```python
from build123d import *

# Parameters (mm, degrees)
SKETCH1_W                       = 100
SKETCH1_H                       = 270
BOSS_EXTRUDE1_DEPTH             = 20
M8_TAPPED_HOLE1_D               = 6.8
M8_TAPPED_HOLE1_DEPTH           = 19.75
M8_TAPPED_HOLE1_TIP             = 2.042926105
M8_TAPPED_HOLE1_ON_FACE_2_D     = 6.8
M8_TAPPED_HOLE1_ON_FACE_2_DEPTH = 19.75
M8_TAPPED_HOLE1_ON_FACE_2_TIP   = 2.042926105
M4_TAPPED_HOLE2_D               = 3.3
M4_TAPPED_HOLE2_DEPTH           = 10.1
M4_TAPPED_HOLE2_TIP             = 0.991420021
M4_TAPPED_HOLE1_D               = 3.3
M4_TAPPED_HOLE1_DEPTH           = 10.1
M4_TAPPED_HOLE1_TIP             = 0.991420021


with BuildPart() as part:
    # Sketch1 → Boss-Extrude1 (new body)
    with BuildSketch(Plane.XY):
        with Locations((50, -135)):
            Rectangle(SKETCH1_W, SKETCH1_H)
    extrude(amount=BOSS_EXTRUDE1_DEPTH)

    # M8 Tapped Hole1
    with Locations(Plane(origin=(15, 0, 10), x_dir=(0, 0, 1), z_dir=(0, 1, 0))):
        with Locations((0, 0), (0, 70)):
            Hole(M8_TAPPED_HOLE1_D / 2, depth=M8_TAPPED_HOLE1_DEPTH)
            with Locations((0, 0, -(M8_TAPPED_HOLE1_DEPTH + M8_TAPPED_HOLE1_TIP / 2))):  # 118° drill point
                Cone(0, M8_TAPPED_HOLE1_D / 2, M8_TAPPED_HOLE1_TIP, mode=Mode.SUBTRACT)

    # M8 Tapped Hole1 on face 2
    with Locations(Plane(origin=(15, -270, 10), x_dir=(0, 0, -1), z_dir=(0, -1, 0))):
        with Locations((0, 0), (0, 70)):
            Hole(M8_TAPPED_HOLE1_ON_FACE_2_D / 2, depth=M8_TAPPED_HOLE1_ON_FACE_2_DEPTH)
            with Locations((0, 0, -(M8_TAPPED_HOLE1_ON_FACE_2_DEPTH + M8_TAPPED_HOLE1_ON_FACE_2_TIP / 2))):  # 118° drill point
                Cone(0, M8_TAPPED_HOLE1_ON_FACE_2_D / 2, M8_TAPPED_HOLE1_ON_FACE_2_TIP, mode=Mode.SUBTRACT)

    # M4 Tapped Hole2
    with Locations(Plane.XY.offset(20)):
        with Locations((50, -127.5), (50, -142.5)):
            Hole(M4_TAPPED_HOLE2_D / 2, depth=M4_TAPPED_HOLE2_DEPTH)
            with Locations((0, 0, -(M4_TAPPED_HOLE2_DEPTH + M4_TAPPED_HOLE2_TIP / 2))):  # 118° drill point
                Cone(0, M4_TAPPED_HOLE2_D / 2, M4_TAPPED_HOLE2_TIP, mode=Mode.SUBTRACT)

    # M4 Tapped Hole1
    with Locations(Plane(origin=(0, 0, 0), x_dir=(-1, 0, 0), z_dir=(0, 0, -1))):
        with Locations((-60, -55), (-60, -115), (-60, -175)):
            Hole(M4_TAPPED_HOLE1_D / 2, depth=M4_TAPPED_HOLE1_DEPTH)
            with Locations((0, 0, -(M4_TAPPED_HOLE1_DEPTH + M4_TAPPED_HOLE1_TIP / 2))):  # 118° drill point
                Cone(0, M4_TAPPED_HOLE1_D / 2, M4_TAPPED_HOLE1_TIP, mode=Mode.SUBTRACT)


solid = part.part
```
Work out the finished part from the listing and answer in its coordinate system (mm). A direction names the side the tool comes from. Round coordinates to 2 decimals unless told otherwise and drop trailing zeros. Return JSON: item names as keys, results as strings. Group by question number.
Q1. Find the intervals of material crossed by L1, parallel to X at y = -14.75, z = 10; L2, parallel to Y at x = 50, z = 17; L3, parallel to X at y = -127.5, z = 17.5, in increasing order.
Q2. For faces 1 (the flat face through (49, -133, 0)), 2 (the cylindrical face through (81.68, -10.01, 10.74)), 3 (the cylindrical face through (81.68, -259.99, 9.26)), determine the directions among +Z, -Z, +X, -X, +Y, -Y from which every point of the face is accessible in a straight line to the end or side of a thin tool.
Q3. Each of these flat-tipped pins is pushed along its axis until it touches: pin 1 Ø4 at (x, z) = (85, 10) entering from -Y; pin 2 Ø6 at (x, z) = (15, 10) entering from -Y; pin 3 Ø2.5 at (x, y) = (60, -175) entering from -Z. Where does it stop, or does it pass through?
Q4. The mould has two halves that part along X. Classify faces 4 (the flat face through (49, -133, 20)), 5 (the cylindrical face through (12, -10, 8.4)), 6 (the flat face through (100, -137, 10)): released by +X, released by -X, zero draft, split by the parting line, or undercut.
Solved:
{
 "1": {"L1": "0 to 11.6, 18.4 to 81.6, 88.4 to 100", "L2": "-270 to -144.15, -140.85 to -129.15, -125.85 to 0", "L3": "0 to 48.35, 51.65 to 100"},
 "2": {"face 1": "-Z, +X, -X, +Y, -Y", "face 2": "+Y", "face 3": "-Y"},
 "3": {"pin 1": "y = -249.41", "pin 2": "y = -250.01", "pin 3": "z = 10.34"},
 "4": {"face 4": "zero draft", "face 5": "undercut", "face 6": "released by +X"}
}
